Read the model definition and answer for the solid it produces. Units are mm, in the model's axes. A direction names the side the tool comes from. Give positions to 0.01 mm unless a question says otherwise; leave off trailing zeros. Loops run counter-clockwise (first coordinate to the right, second up) from the corner with the lowest first, then second, coordinate; pieces in that order, holes last.
(1) Find section B-B, the plane z = -20. Write down the section's boundary in (x, y).
(2) Find section C-C, the plane x = 100. Write down the section's boundary in (y, z).
(3) Find section A-A, the plane y = 70. Write down the section's boundary in (x, z), then the cut area to 3 significant figures.
(4) Determine the mould class of faces 5 (the face through (0, 15, -12)), 6 (the face through (85, 40, -80)), 7 (the face through (100, 52, -65)) for opening direction Z: pulls with the +Z half, pulls with the -Z half, needs draft (parallel to the pull), parting line crosses it, or undercut.
(5) Find section D-D, the plane y = 12. Write down the section's boundary in (x, z).
(6) Which of the six approach directions +Z, -Z, +X, -X, +Y, -Y give full straight-line access (tool end or side, diameter ignored) to faces 1 (the face through (100, 52, -15)), 2 (the face through (67, 82, -25)), 3 (the face through (43, 30, -48)), 4 (the face through (85, 10, -39))?
(7) Each of these flat-tipped pins is pushed along its axis until it touches: P1, Ø2, axis at y = 63, z = -22.5, coming from the -X side; P2, Ø6, axis at x = 68.5, z = -22.5, coming from the -Y side; P3, Ø16.5, axis at x = 95.5, z = -10, coming from the -Y side; P4, Ø18, axis at x = 37, z = -57.5, coming from the +Y side. Where does it stop, or does it pass through?
(8) Straight lines are drawn through the part: probe 1 along Z at (x, y) = (71.5, 88); probe 2 along Z at (x, y) = (84, 27.5); probe 3 along Y at (x, z) = (100, -5.25). For each, find the intervals that lie inside material, in ascending order.
```python
from build123d import *

# Parameters (mm, degrees)
BASE_BLOCK_SKETCH_W             = 140
BASE_BLOCK_SKETCH_H             = 30
BASE_BLOCK_DEPTH                = 80
BASE_NOTCH_SKETCH_W             = 40
BASE_NOTCH_SKETCH_H             = 20
BASE_NOTCH_DEPTH                = 80
UPRIGHT_SKETCH_W                = 80
UPRIGHT_SKETCH_H                = 70
UPRIGHT_DEPTH                   = 80
UPRIGHT_PROFILE_CUT_DEPTH       = 80
CROSS_HOLE_SKETCH_R             = 15
CROSS_HOLE_DEPTH                = 80
UPRIGHT_U_SLOT_DEPTH            = 80
BASE_UNDERSIDE_NOTCH_DEPTH      = 10
BASE_UNDERSIDE_NOTCH_DEPTH_BACK = 80


with BuildPart() as part:
    # Base Block Sketch → Base Block (new body)
    with BuildSketch(Plane.XY):
        with Locations((70, 15)):
            Rectangle(BASE_BLOCK_SKETCH_W, BASE_BLOCK_SKETCH_H)
    extrude(amount=-BASE_BLOCK_DEPTH)

    # Base Notch Sketch → Base Notch (cut)
    with BuildSketch(Plane.XY):
        with Locations((105, 10)):
            Rectangle(BASE_NOTCH_SKETCH_W, BASE_NOTCH_SKETCH_H)
    extrude(amount=-BASE_NOTCH_DEPTH, mode=Mode.SUBTRACT)

    # Upright Sketch → Upright (add)
    with BuildSketch(Plane.XY):
        with Locations((100, 65)):
            Rectangle(UPRIGHT_SKETCH_W, UPRIGHT_SKETCH_H)
    extrude(amount=-UPRIGHT_DEPTH)

    # Upright Profile Cut Sketch → Upright Profile Cut (cut)
    with BuildSketch(Plane(origin=(0, 100, 0), x_dir=(1, 0, 0), z_dir=(0, 1, 0))):
        Polygon((75, 15), (75, 40), (75, 65), (125, 65), (125, 15), align=None)
    extrude(amount=-UPRIGHT_PROFILE_CUT_DEPTH, mode=Mode.SUBTRACT)

    # Cross Hole Sketch → Cross Hole (cut)
    with BuildSketch(Plane.XY):
        with Locations((100, 70)):
            Circle(CROSS_HOLE_SKETCH_R)
    extrude(amount=-CROSS_HOLE_DEPTH, mode=Mode.SUBTRACT)

    # Upright U-Slot Sketch → Upright U-Slot (cut)
    with BuildSketch(Plane.ZY.offset(-60)):
        with BuildLine():
            Line((-25, 100), (-55, 100))
            Line((-55, 100), (-55, 65))
            ThreePointArc((-55, 65), (-40, 50), (-25, 65))
            Line((-25, 65), (-25, 100))
        make_face()
    extrude(amount=-UPRIGHT_U_SLOT_DEPTH, mode=Mode.SUBTRACT)

    # Base Underside Notch Sketch → Base Underside Notch (cut, two sides: drawn at the far end of the back side and taken through both)
    with BuildSketch(Plane(origin=(0, 30, 0), x_dir=(1, 0, 0), z_dir=(0, 1, 0)).offset(-BASE_UNDERSIDE_NOTCH_DEPTH_BACK)):
        with BuildLine():
            Line((30, 55), (0, 55))
            Line((0, 55), (0, 25))
            Line((0, 25), (30, 25))
            ThreePointArc((30, 25), (45, 40), (30, 55))
        make_face()
    extrude(amount=BASE_UNDERSIDE_NOTCH_DEPTH + BASE_UNDERSIDE_NOTCH_DEPTH_BACK, mode=Mode.SUBTRACT)


solid = part.part
```
Entries:
1. outline: (0, 0) - (85, 0) - (85, 20) - (75, 20) - (75, 100) - (60, 100) - (60, 30) - (0, 30) - close; (125, 0) - (140, 0) - (140, 100) - (125, 100) - close
2. outline: (20, -80) - (55, -80) - (55, -65) - (20, -65) - close; (20, -15) - (55, -15) - (55, 0) - (20, 0) - close; (85, -80) - (100, -80) - (100, -65) - (85, -65) - close; (85, -15) - (100, -15) - (100, 0) - (85, 0) - close
3. outline: (60, -80) - (85, -80) - (85, -65) - (75, -65) - (75, -55) - (60, -55) - close; (60, -25) - (75, -25) - (75, -15) - (85, -15) - (85, 0) - (60, 0) - close; (115, -80) - (140, -80) - (140, -55) - (125, -55) - (125, -65) - (115, -65) - close; (115, -15) - (125, -15) - (125, -25) - (140, -25) - (140, 0) - (115, 0) - close
3. area: 2,100 mm2
4. face 5: needs draft
4. face 6: pulls with the -Z half
4. face 7: undercut
5. outline: (0, -80) - (85, -80) - (85, 0) - (0, 0) - (0, -25) - (30, -25) arc R15 cw to (30, -55) - (0, -55) - close; (125, -80) - (140, -80) - (140, 0) - (125, 0) - close
6. face 1: +Y
6. face 2: +X, -X, +Y
6. face 3: +Z, -Z, -X, +Y
6. face 4: +Z, -Z, -Y
7. P1: stops at x = 60
7. P2: stops at y = 0
7. P3: stops at y = 20
7. P4: stops at y = 30
8. probe 1: z = -80 to -55, -25 to 0
8. probe 2: z = -80 to -65, -15 to 0
8. probe 3: y = 20 to 55, 85 to 100
